Here's how the part is built. I have some questions about the finished solid (model axes, mm). A direction names the side the tool comes from. Round coordinates to 2 decimals unless told otherwise and drop trailing zeros. Write each loop counter-clockwise with the first axis right and the second up, starting at its lowest first coordinate (ties: lowest second). Pieces come first, ordered by that corner, then holes. Notation, with made-up numbers: (-16.5, 40) -> (12.5, 40) arc R25 ccw to (12.5, 76) -> close; hole circle Ø10 at (-15, 33). An arc over 180 degrees is marked (long way). Answer as CSV lines item,"result".
from build123d import *

# Parameters (mm, degrees)
BOSS_EXTRUDE1_DEPTH    = 60
CHAMFER1_SIZE          = 10
M18_TAPPED_HOLE1_D     = 15.5
M18_TAPPED_HOLE1_DEPTH = 43.5
M18_TAPPED_HOLE1_TIP   = 4.656669797


with BuildPart() as part:
    # Sketch1 → Boss-Extrude1 (new body)
    with BuildSketch(Plane.XY):
        with BuildLine():
            Line((0, 0), (95, 0))
            ThreePointArc((95, 0), (105.606601718, -4.393398282), (110, -15))
            Line((110, -15), (110, -67))
            Line((110, -67), (100, -67))
            Line((100, -67), (100, -15))
            ThreePointArc((100, -15), (98.535533906, -11.464466094), (95, -10))
            Line((95, -10), (0, -10))
            Line((0, -10), (0, 0))
        make_face()
    extrude(amount=BOSS_EXTRUDE1_DEPTH)

    # Chamfer1
    chamfer1_edges = [part.edges().sort_by_distance(p)[0] for p in [
        (0, -5, 0),
        (0, -5, 60),
    ]]
    chamfer(chamfer1_edges, length=CHAMFER1_SIZE)

    # M18 Tapped Hole1
    with Locations(Plane(origin=(0, 0, 0), x_dir=(1, 0, 0), z_dir=(0, 1, 0))):
        with Locations((25, -30)):
            Hole(M18_TAPPED_HOLE1_D / 2, depth=M18_TAPPED_HOLE1_DEPTH)
            with Locations((0, 0, -(M18_TAPPED_HOLE1_DEPTH + M18_TAPPED_HOLE1_TIP / 2))):  # 118° drill point
                Cone(0, M18_TAPPED_HOLE1_D / 2, M18_TAPPED_HOLE1_TIP, mode=Mode.SUBTRACT)


solid = part.part
Item 1: Suppose I cut it at D-D, the plane x = 77. List the corners of the cut face in (y, z) for me.
Results found:
outline,"(-10, 0) -> (0, 0) -> (0, 60) -> (-10, 60) -> close"
Item 2: I need wall thicknesses on L1, parallel to Z at x = 25, y = -2.25; L2, parallel to X at y = -54, z = 23.5; L3, parallel to Y at x = 73.5, z = 49.5. Which ranges of each line are inside material? Lowest first, please.
Results found:
L1,"z = 0 to 22.25, 37.75 to 60"
L2,"x = 100 to 110"
L3,"y = -10 to 0"
Item 3: Suppose I cut it at B-B, the plane x = 25. List the corners of the cut face in (y, z) for me.
Results found:
outline,"(-10, 0) -> (0, 0) -> (0, 22.25) -> (-10, 22.25) -> close; (-10, 37.75) -> (0, 37.75) -> (0, 60) -> (-10, 60) -> close"
Item 4: Will these pins go through, and if not, where does the flat tip stop? pin 1 (2 mm diameter, centred on y = -13, z = 51.5, fed in from -X); pin 2 (10 mm diameter, centred on x = 85, z = 51.5, fed in from -Y); pin 3 (15.5 mm diameter, centred on y = -30, z = 17, fed in from -X).
Results found:
pin 1,"stops at x = 99"
pin 2,"stops at y = -10"
pin 3,"stops at x = 100"
Item 5: If we mould it in two halves opening along X, with no side actions, what happens to faces 1 (the flat face through (79, -9, 60)), 2 (the cylindrical face through (20.834, -5.07, 23.465)), 3 (the cylindrical face through (99, -12, 30))? For each: pulls with the +X half, pulls with the -X half, needs draft (parallel to the pull), parting line crosses it, or undercut.
Results found:
face 1,"needs draft"
face 2,"undercut"
face 3,"pulls with the -X half"
Item 6: For faces 4 (the flat face through (110, -41, 30)), 5 (the flat face through (100, -41, 30)), which set-ups out of +Z, -Z, +X, -X, +Y, -Y let a thin tool reach every point of the face, with its end or its side?
Results found:
face 4,"+Z, -Z, +X, +Y, -Y"
face 5,"+Z, -Z, -X, -Y"
Item 7: Suppose I cut it at A-A, the plane z = 30. List the corners of the cut face in (x, y) for me.
Results found:
outline,"(0, -10) -> (17.25, -10) -> (17.25, 0) -> (0, 0) -> close; (32.75, -10) -> (95, -10) arc R5 cw to (100, -15) -> (100, -67) -> (110, -67) -> (110, -15) arc R15 ccw to (95, 0) -> (32.75, 0) -> close"
Item 8: Suppose I cut it at C-C, the plane z = 12. List the corners of the cut face in (x, y) for me.
Results found:
outline,"(0, -10) -> (95, -10) arc R5 cw to (100, -15) -> (100, -67) -> (110, -67) -> (110, -15) arc R15 ccw to (95, 0) -> (0, 0) -> close"
